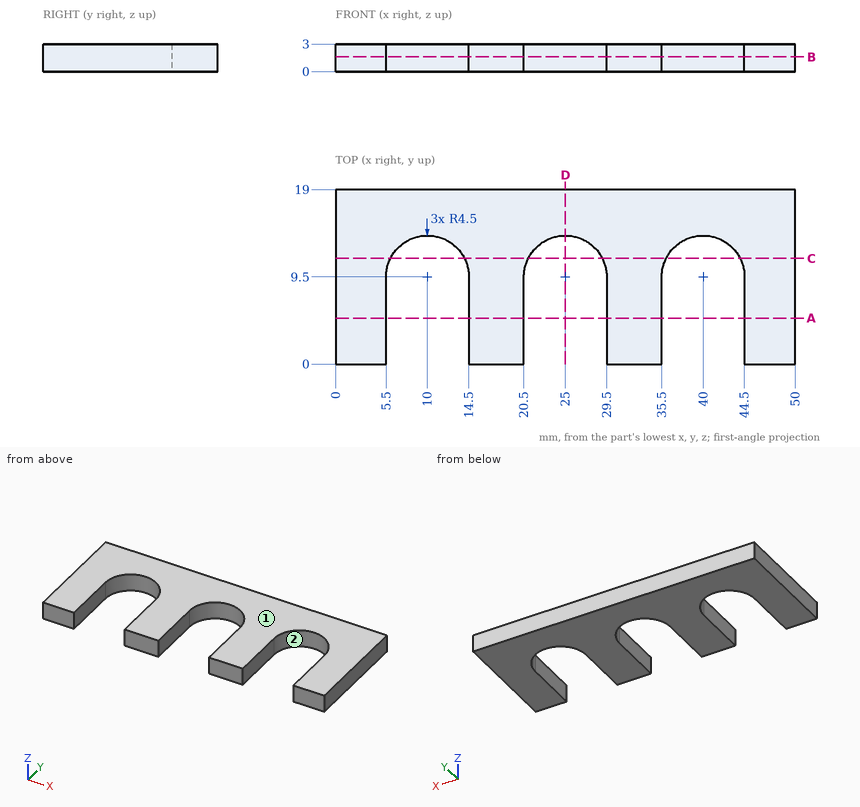
For this review, use the dimensioned drawing (mm, ordinates from the lowest corner) and the shaded views. Give positions to 0.01 mm unless a question says otherwise; leave off trailing zeros. Order: outer loops, then holes, each group sorted by start corner. A loop starts at its lowest first (then second) coordinate and runs counter-clockwise, first axis right, second up.
1) The part is to be moulded in two halves that separate along X. For the marked faces 1 and 2, say which applies: released by +X, released by -X, zero draft, split by the parting line, or undercut.
2) Take a section at B-B (z = 1.6). Give the boundary of the cut face in (x, y).
3) Take a section at D-D (x = 25). Give the boundary of the cut face in (y, z), then the cut area to 3 significant figures.
4) Wall thickness on line 1 (X direction, y = 3.5, z = 1.05); line 2 (X direction, y = 11.5, z = 0.55); line 3 (Y direction, x = 39.5, z = 1.85): over which ranges is each line inside the solid? List them lowest first.
5) Take a section at C-C (y = 11.5). Give the boundary of the cut face in (x, z), then the cut area to 3 significant figures.
6) Take a section at A-A (y = 5). Give the boundary of the cut face in (x, z), then the cut area to 3 significant figures.
Derived:
1. face 1: zero draft
1. face 2: undercut
2. outline: (0, 0) - (5.5, 0) - (5.5, 9.5) arc R4.5 cw to (14.5, 9.5) - (14.5, 0) - (20.5, 0) - (20.5, 9.5) arc R4.5 cw to (29.5, 9.5) - (29.5, 0) - (35.5, 0) - (35.5, 9.5) arc R4.5 cw to (44.5, 9.5) - (44.5, 0) - (50, 0) - (50, 19) - (0, 19) - close
3. outline: (14, 0) - (19, 0) - (19, 3) - (14, 3) - close
3. area: 15.0 mm2
4. line 1: x = 0 to 5.5, 14.5 to 20.5, 29.5 to 35.5, 44.5 to 50
4. line 2: x = 0 to 5.97, 14.03 to 20.97, 29.03 to 35.97, 44.03 to 50
4. line 3: y = 13.97 to 19
5. outline: (0, 0) - (5.97, 0) - (5.97, 3) - (0, 3) - close; (14.03, 0) - (20.97, 0) - (20.97, 3) - (14.03, 3) - close; (29.03, 0) - (35.97, 0) - (35.97, 3) - (29.03, 3) - close; (44.03, 0) - (50, 0) - (50, 3) - (44.03, 3) - close
5. area: 77.4 mm2
6. outline: (0, 0) - (5.5, 0) - (5.5, 3) - (0, 3) - close; (14.5, 0) - (20.5, 0) - (20.5, 3) - (14.5, 3) - close; (29.5, 0) - (35.5, 0) - (35.5, 3) - (29.5, 3) - close; (44.5, 0) - (50, 0) - (50, 3) - (44.5, 3) - close
6. area: 69.0 mm2
